Build history of the part. All positions in model axes, mm. A direction names the side the tool comes from. Round coordinates to 2 decimals unless told otherwise and drop trailing zeros. Loops run counter-clockwise (first coordinate to the right, second up) from the corner with the lowest first, then second, coordinate; pieces in that order, holes last. Notation, with made-up numbers: (-4, 27.25) - (20, 27.25) arc R28 ccw to (20, 55.25) - close; hole circle Ø1 at (19, -30). An arc over 180 degrees is marked (long way). Use a Markdown table: item, result.
from build123d import *

# Parameters (mm, degrees)
BOSS_EXTRUDE1_DEPTH     = 50
SKETCH2_W               = 15
SKETCH2_H               = 30
CUT_EXTRUDE1_DEPTH      = 20
CUT_EXTRUDE2_DEPTH      = 594.131240453
CUT_EXTRUDE2_DEPTH_BACK = 594.131240453
FILLET1_R               = 3


with BuildPart() as part:
    # Sketch1 → Boss-Extrude1 (new body)
    with BuildSketch(Plane.XY):
        with BuildLine():
            Line((-307.585956352, 341.88779966), (-311.885113994, 384.650908092))
            ThreePointArc((-311.885113994, 384.650908092), (-387.611395489, 361.512211901), (-448.718561356, 311.155650759))
            Line((-448.718561356, 311.155650759), (-415.440513877, 283.957530324))
            ThreePointArc((-415.440513877, 283.957530324), (-367.274758623, 323.649467677), (-307.585956352, 341.88779966))
        make_face()
    extrude(amount=BOSS_EXTRUDE1_DEPTH)

    # Sketch2 → Cut-Extrude1 (cut)
    with BuildSketch(Plane(origin=(-237.484086125, 442.147798063, 0), x_dir=(0.880965905900498, 0.47317974665122253, 0), z_dir=(-0.47317974665122253, 0.880965905900498, 0))):
        with Locations((-222.912167325, -28)):
            Rectangle(SKETCH2_W, SKETCH2_H)
        with Locations((-117.912167325, -28)):
            Rectangle(SKETCH2_W, SKETCH2_H)
    extrude(amount=-CUT_EXTRUDE1_DEPTH, mode=Mode.SUBTRACT)

    # Sketch3 → Cut-Extrude2 (cut, two sides: drawn at the far end of the back side and taken through both)
    with BuildSketch(Plane(origin=(0, 0, 0), x_dir=(-1, 0, 0), z_dir=(0, 0, -1)).offset(-CUT_EXTRUDE2_DEPTH_BACK)):
        with BuildLine():
            ThreePointArc((403.644999576, 345.361735137), (385.937282785, 356.235559249), (367.185078684, 365.188666312))
            ThreePointArc((367.185078684, 365.188666312), (357.385414117, 361.130763607), (361.443316822, 351.33109904))
            ThreePointArc((361.443316822, 351.33109904), (378.77130289, 343.057974791), (395.134129798, 333.010010739))
            ThreePointArc((395.134129798, 333.010010739), (405.565426886, 334.930438049), (403.644999576, 345.361735137))
        make_face()
    extrude(amount=CUT_EXTRUDE2_DEPTH + CUT_EXTRUDE2_DEPTH_BACK, mode=Mode.SUBTRACT)

    # Fillet1
    fillet1_edges = [part.edges().sort_by_distance(p)[0] for p in [
        (-387.611395489, 361.512211901, 50),
        (-432.079537616, 297.556590541, 50),
        (-367.274758623, 323.649467677, 50),
        (-432.079537616, 297.556590541, 0),
        (-387.611395489, 361.512211901, 0),
        (-309.735535173, 363.269353876, 0),
        (-367.274758623, 323.649467677, 0),
        (-415.440513877, 283.957530324, 25),
        (-448.718561356, 311.155650759, 25),
        (-311.885113994, 384.650908092, 25),
        (-307.585956352, 341.88779966, 25),
        (-309.735535173, 363.269353876, 50),
    ]]
    fillet(fillet1_edges, radius=FILLET1_R)


solid = part.part
Q1. Pull direction X, two halves, no side cores. Call faces 5 (the face through (-378, 335, 0)), 6 (the face through (-378.53, 343.19, 25.35)), 7 (the face through (-342.09, 371.86, 28.21)), 8 (the face through (-310.61, 363.42, 0.9)): pulls with the +X half, pulls with the -X half, needs draft (parallel to the pull), parting line crosses it, or undercut.
Results found:
| item | result |
|---|---|
| face 5 | needs draft |
| face 6 | undercut |
| face 7 | undercut |
| face 8 | pulls with the +X half |
Q2. Drop flat-ended pins along their axis: pin 1 (3 mm diameter, centred on y = 344.5, z = 29.5, fed in from -X); pin 2 (3 mm diameter, centred on x = -391.5, z = 23, fed in from +Y); pin 3 (10 mm diameter, centred on x = -389.5, z = 15, fed in from -Y). Give the stop position or say it passes through.
Results found:
| item | result |
|---|---|
| pin 1 | stops at x = -416.07 |
| pin 2 | stops at y = 360.21 |
| pin 3 | stops at y = 305.19 |
Q3. Probe line 1 (X direction, y = 355, z = 34.5); line 2 (Y direction, x = -328, z = 32); line 3 (X direction, y = 345, z = 46). List the from-to ranges inside material, lowest first.
Results found:
| item | result |
|---|---|
| line 1 | x = -398.86 to -388.17, -357.56 to -308.9 |
| line 2 | y = 338.49 to 370.83, 377.33 to 382.37 |
| line 3 | x = -413.46 to -404.13, -375.1 to -307.9 |
Q4. Which spindle directions (+Z, -Z, +X, -X, +Y, -Y) get a long thin tool onto all of the face, cutting with end or side? Do faces 1 (the face through (-386.19, 356.1, 25.35)), 2 (the face through (-432.261, 297.705, 24.692)), 3 (the face through (-433.627, 320.383, 28.21)), 4 (the face through (-421.38, 329.28, 28.21)). Say none if no direction does.
Results found:
| item | result |
|---|---|
| face 1 | +Z, -Z |
| face 2 | +Z, -Z, -X, -Y |
| face 3 | +Y |
| face 4 | none |
Q5. Cut at A-A, the plane z = 29.5. List the corners of the cut face in (x, y) (3 decimals), plus the area to 3 significant figures.
Results found:
| item | result |
|---|---|
| outline | (-446.774, 313.499) arc R3 ccw to (-446.378, 309.243) - (-417.742, 285.839) arc R3 ccw to (-413.556, 286.22) arc R159.959 cw to (-310.513, 341.566) arc R3 ccw to (-307.883, 344.845) - (-311.583, 381.644) arc R3 ccw to (-314.913, 384.324) arc R202.938 ccw to (-330.461, 381.91) - (-325.29, 372.284) - (-338.504, 365.186) - (-345.577, 378.355) arc R202.938 ccw to (-424.864, 335.768) - (-417.791, 322.6) - (-431.006, 315.502) - (-436.176, 325.129) arc R202.938 ccw to start; hole (-403.645, 345.362) arc R7.5 ccw to (-395.134, 333.01) arc R182.5 cw to (-361.443, 351.331) arc R7.5 ccw to (-367.185, 365.189) arc R197.5 ccw to start |
| area | 4,950 mm2 |
